Here's how the part is built. I have some questions about the finished solid (model axes, mm). Face numbers are marked on the shaded views. Round coordinates to 2 decimals unless told otherwise and drop trailing zeros. Write each loop counter-clockwise with the first axis right and the second up, starting at its lowest first coordinate (ties: lowest second). Pieces come first, ordered by that corner, then holes. Notation, with made-up numbers: (24.5, -26.5) - (39.5, -26.5) arc R18 cw to (39.5, -21.5) - close; hole circle Ø9 at (53, 65.25). An arc over 180 degrees is marked (long way). Write item = value, one per line. Start each with the question number.
Item 1: If we section it at B-B (z = 10): Please give me the cut outline in (x, y), and give its area (3 significant figures).
Item 2: Thinking about a two-plate mould opening in X: for the marked faces 1, 2, 3 and 4, which applies, pulls with the +X half, pulls with the -X half, needs draft (parallel to the pull), parting line crosses it, or undercut?
Item 3: For P1, Ø12, axis at y = -3.5, z = 3, coming from the +X side; P2, Ø1.5, axis at y = 3, z = 16, coming from the +X side; P3, Ø1, axis at x = 27.5, y = 4, coming from the +Z side, each with a flat end and sliding along its axis, tell me the tip position at first contact or that it passes through.
Item 4: If I drill on line 1 along Y through (x, z) = (0, 10.5); line 2 along Y through (x, z) = (65, 7); line 3 along X through (y, z) = (-20.5, 8.75), over which ranges is the centre line in solid material (lowest first)? Write a range as [from, to].
Item 5: If we section it at A-A (x = -12): Please give me the cut outline in (y, z), and give its area (3 significant figures).
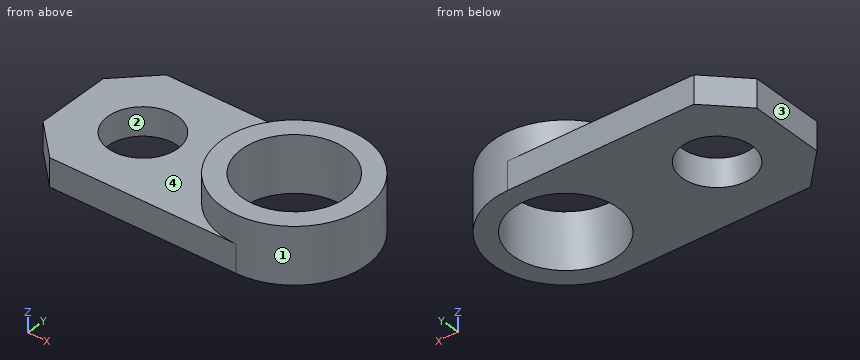
```python
from build123d import *

# Parameters (mm, degrees)
BASE_PLATE_DEPTH = 12
BOSS_SKETCH_62_R = 31
BOSS_62_DEPTH    = 12
BORE_SKETCH_45_R = 22.5
BORE_45_DEPTH    = 25
HOLE_SKETCH_30_R = 15
HOLE_30_DEPTH    = 25


with BuildPart() as part:
    # Base Plate Sketch → Base Plate (new body)
    with BuildSketch(Plane.XY):
        with BuildLine():
            Line((-15, -31), (65, -31))
            ThreePointArc((65, -31), (96, 0), (65, 31))
            Line((65, 31), (-15, 31))
            Line((-15, 31), (-30, 16))
            Line((-30, 16), (-30, 0))
            Line((-30, 0), (-30, -16))
            Line((-30, -16), (-15, -31))
        make_face()
    extrude(amount=BASE_PLATE_DEPTH)

    # Boss Sketch Ø62 → Boss Ø62 (add)
    with BuildSketch(Plane.XY.offset(12)):
        with Locations(Location((65, 0, 0), (0, 0, 90))):
            Circle(BOSS_SKETCH_62_R)
    extrude(amount=BOSS_62_DEPTH)

    # Bore Sketch Ø45 → Bore Ø45 (cut)
    with BuildSketch(Plane.XY.offset(24)):
        with Locations((65, 0)):
            Circle(BORE_SKETCH_45_R)
    extrude(amount=-BORE_45_DEPTH, mode=Mode.SUBTRACT)

    # Hole Sketch Ø30 → Hole Ø30 (cut)
    with BuildSketch(Plane.XY.offset(12)):
        Circle(HOLE_SKETCH_30_R)
    extrude(amount=-HOLE_30_DEPTH, mode=Mode.SUBTRACT)


solid = part.part
```
Reply:
q1.outline = (-30, -16) - (-15, -31) - (65, -31) arc R31 ccw to (65, 31) - (-15, 31) - (-30, 16) - close; hole circle Ø30 at (0, 0); hole circle Ø45 at (65, 0)
q1.area = 4,880 mm2
q2.face_1 = parting line crosses it
q2.face_2 = undercut
q2.face_3 = pulls with the -X half
q2.face_4 = needs draft
q3.P1 = 96
q3.P2 = 95.92
q3.P3 = 12
q4.line_1 = [-31, -15], [15, 31]
q4.line_2 = [-31, -22.5], [22.5, 31]
q4.line_3 = [-25.5, 55.73], [74.27, 88.25]
q5.outline = (-31, 0) - (-9, 0) - (-9, 12) - (-31, 12) - close; (9, 0) - (31, 0) - (31, 12) - (9, 12) - close
q5.area = 528 mm2
